Here's the drawing with two shaded views (mm, measured from the low corner). I have some questions. Give positions to 0.01 mm unless a question says otherwise; leave off trailing zeros. Loops run counter-clockwise (first coordinate to the right, second up) from the corner with the lowest first, then second, coordinate; pieces in that order, holes last. Notation, with made-up numbers: (2.25, -14) -> (41.25, -14) arc R26 cw to (41.25, 24) -> close; hole circle Ø3 at (66, 64.5). An arc over 180 degrees is marked (long way). Write each question's results on one line, items separated by ' | '. Start each with the question number.
Q1. If we section it at A-A, the plane z = 0.7: List the corners of the cut face in (x, y) for me.
Q2. If we section it at C-C, the plane y = 23.5: List the corners of the cut face in (x, z) for me.
Q3. If I drill on line 1 along Y through (x, z) = (48.5, 0.5); line 2 along Y through (x, z) = (15.5, 0.4); line 3 along X through (y, z) = (8, 0.2), over which ranges is the centre line in solid material (lowest first)?
Q4. If we section it at B-B, the plane x = 29: List the corners of the cut face in (y, z) for me, plus the area to 3 significant figures.
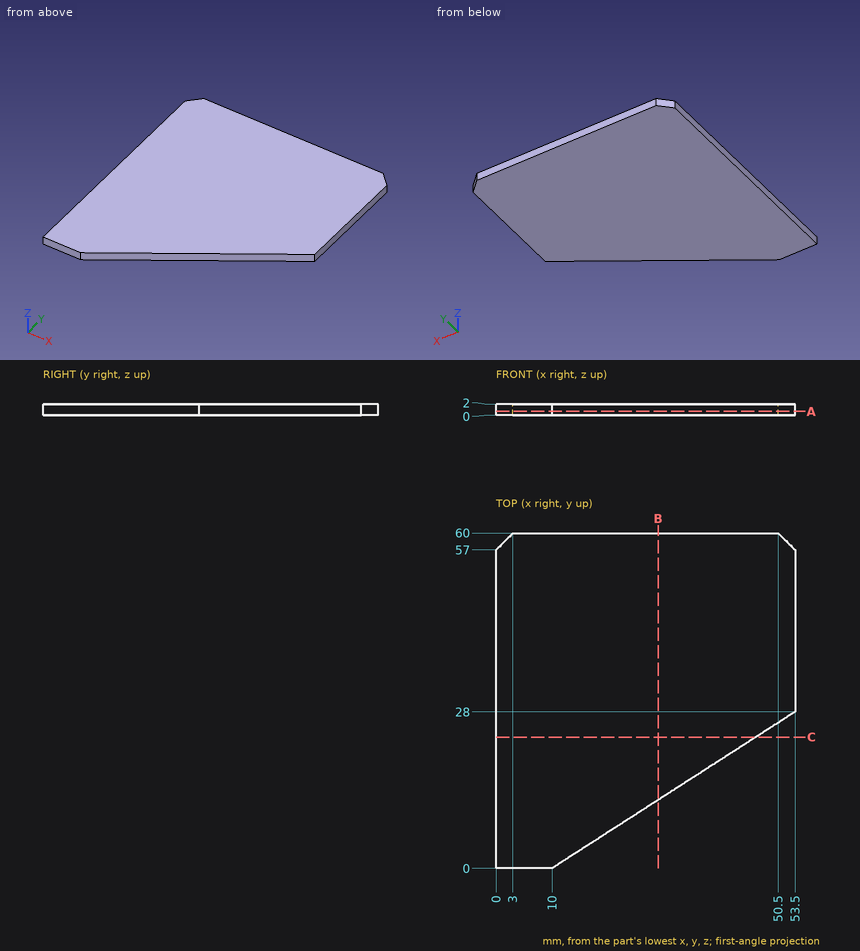
Final values:
1) outline: (0, 0) -> (10, 0) -> (53.5, 28) -> (53.5, 57) -> (50.5, 60) -> (3, 60) -> (0, 57) -> close
2) outline: (0, 0) -> (46.51, 0) -> (46.51, 2) -> (0, 2) -> close
3) line 1: y = 24.78 to 60 | line 2: y = 3.54 to 60 | line 3: x = 0 to 22.43
4) outline: (12.23, 0) -> (60, 0) -> (60, 2) -> (12.23, 2) -> close | area: 95.5 mm²
